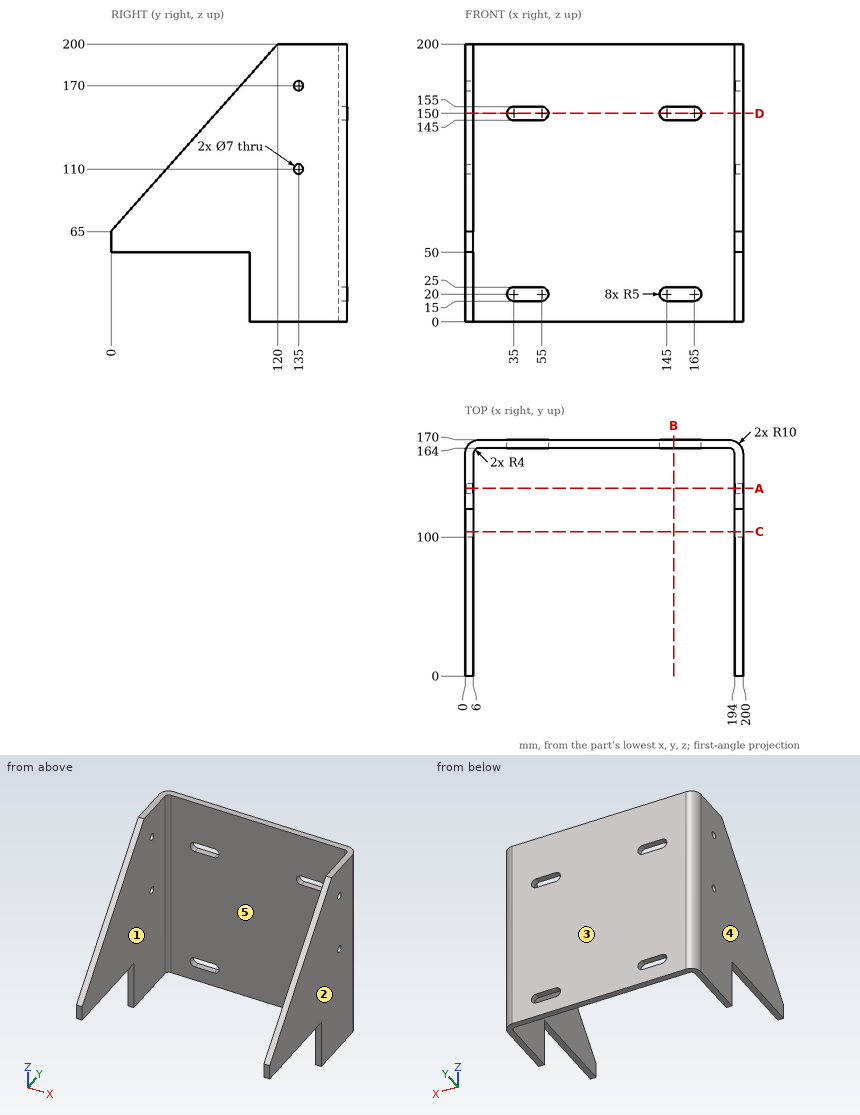
Could you check a few things on this drawing? It's one solid part, dimensions in mm from its lowest x, y, z. A direction names the side the tool comes from. Give positions to 0.01 mm unless a question says otherwise; leave off trailing zeros. Loops run counter-clockwise (first coordinate to the right, second up) from the corner with the lowest first, then second, coordinate; pieces in that order, holes last. Notation, with made-up numbers: (35, 51) -> (68, 51) arc R17 ccw to (68, 80) -> close; hole circle Ø6 at (4, 10.5). An arc over 180 degrees is marked (long way). Answer as CSV lines item,"result". Start each with the question number.
(1) If we section it at D-D on z = 150: Write out the boundary of the cut face in (x, y), then the cut area to 3 significant figures.
(2) We'd pull the mould along X, two halves only. Please class the marked faces 3, 4 and 5: released by +X, released by -X, zero draft, split by the parting line, or undercut.
(3) If we section it at A-A on y = 135: Write out the boundary of the cut face in (x, z).
(4) Which directions (+Z, -Z, +X, -X, +Y, -Y) give clear straight access to the entire face, cutting with the end or side of a thin tool? Please do the marked faces 1 and 2.
(5) If we section it at B-B on x = 150: Write out the boundary of the cut face in (y, z).
(6) I need wall thicknesses on probe 1 along X at (y, z) = (104, 38); probe 2 along Z at (x, y) = (196, 135); probe 3 along Y at (x, z) = (125, 36). Which ranges of each line are inside material? Lowest first, please.
(7) I'm going to push flat-ended pins straight in: pin 1 Ø5 at (x, y) = (196, 71) entering from -Z; pin 2 Ø3 at (x, y) = (43.5, 167) entering from -Z; pin 3 Ø1.8 at (x, z) = (198.5, 24) entering from -Y; pin 4 Ø12 at (x, z) = (174, 95.5) entering from -Y. Where does each tip first touch, or does it pass through?
(8) If we section it at C-C on y = 104: Write out the boundary of the cut face in (x, z), then the cut area to 3 significant figures.
Computed:
1,outline,"(0, 75.56) -> (6, 75.56) -> (6, 160) arc R4 cw to (10, 164) -> (30, 164) -> (30, 170) -> (10, 170) arc R10 ccw to (0, 160) -> close; (60, 164) -> (140, 164) -> (140, 170) -> (60, 170) -> close; (170, 164) -> (190, 164) arc R4 cw to (194, 160) -> (194, 75.56) -> (200, 75.56) -> (200, 160) arc R10 ccw to (190, 170) -> (170, 170) -> close"
1,area,"1,870 mm2"
2,face 3,"zero draft"
2,face 4,"released by -X"
2,face 5,"undercut"
3,outline,"(0, 0) -> (6, 0) -> (6, 106.5) -> (0, 106.5) -> close; (0, 113.5) -> (6, 113.5) -> (6, 166.5) -> (0, 166.5) -> close; (0, 173.5) -> (6, 173.5) -> (6, 200) -> (0, 200) -> close; (194, 0) -> (200, 0) -> (200, 106.5) -> (194, 106.5) -> close; (194, 113.5) -> (200, 113.5) -> (200, 166.5) -> (194, 166.5) -> close; (194, 173.5) -> (200, 173.5) -> (200, 200) -> (194, 200) -> close"
4,face 1,"+Z, -Z, -Y"
4,face 2,"+Z, -Z, +X, +Y, -Y"
5,outline,"(164, 0) -> (170, 0) -> (170, 15) -> (164, 15) -> close; (164, 25) -> (170, 25) -> (170, 145) -> (164, 145) -> close; (164, 155) -> (170, 155) -> (170, 200) -> (164, 200) -> close"
6,probe 1,"x = 0 to 6, 194 to 200"
6,probe 2,"z = 0 to 106.5, 113.5 to 166.5, 173.5 to 200"
6,probe 3,"y = 164 to 170"
7,pin 1,"stops at z = 50"
7,pin 2,"stops at z = 0"
7,pin 3,"stops at y = 100"
7,pin 4,"stops at y = 164"
8,outline,"(0, 0) -> (6, 0) -> (6, 182) -> (0, 182) -> close; (194, 0) -> (200, 0) -> (200, 182) -> (194, 182) -> close"
8,area,"2,180 mm2"
